Read the model definition and answer for the solid it produces. Units are mm, in the model's axes. Face numbers are marked on the shaded views. A direction names the side the tool comes from. Coordinates: 2 decimals unless noted, no trailing zeros. Order: outer loops, then holes, each group sorted by start corner. A loop starts at its lowest first (then second) coordinate and runs counter-clockwise, first axis right, second up. Notation, with made-up numbers: (4.25, 85) -> (33.25, 85) arc R20 cw to (33.25, 115) -> close; hole circle Ø10 at (39.25, -27.5). An arc over 180 degrees is marked (long way). Answer in a Markdown table with one row per item.
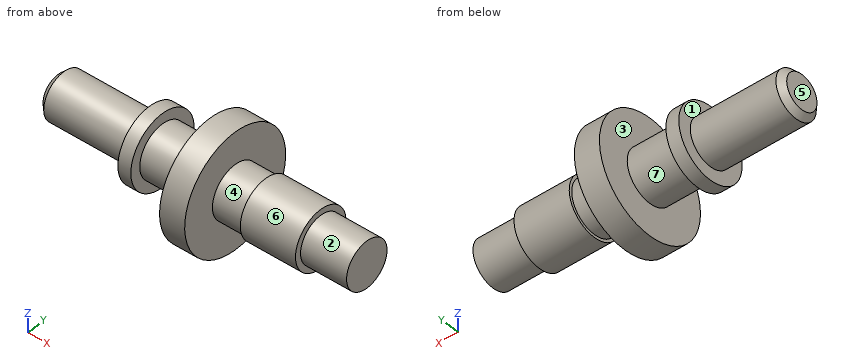
from build123d import *


with BuildPart() as part:
    # Model → Revolve1 (revolve)
    with BuildSketch(Plane.XY, mode=Mode.PRIVATE) as revolve1_sk:
        Polygon((49.51331086, -13.474001866), (49.517097509, -14.469395389), (57.517097509, -14.469395389), (57.517097509, -18.474001866), (3.884490088, -18.474001866), (3.884490088, -15.474001866), (4.884490088, -14.474001866), (11.769027201, -14.474001866), (19.769026262, -14.474001866), (19.769027201, -12.204912355), (22.015056766, -12.204912355), (22.015056766, -13.974001866), (30.280660424, -13.974001866), (30.280660424, -8.474001866), (34.643062355, -8.474001866), (34.643062355, -13.974001866), (39.923864692, -13.974001866), (39.923864692, -13.474001866), align=None)
    revolve(revolve1_sk.sketch.rotate(Axis((3.884490088, -18.474001866, 0), (-1, 0, 0)), 90), axis=Axis((3.884490088, -18.474001866, 0), (-1, 0, 0)))


solid = part.part
Q1. Consider line 1 (X direction, y = -20.75, z = -4.75); line 2 (X direction, y = -25.5, z = -1.75); line 3 (Z direction, x = 12, y = -20.5). Determine where each line is inside the solid, lowest interval first.
Outcome:
| item | result |
|---|---|
| line 1 | 19.77 to 22.02, 30.28 to 34.64 |
| line 2 | 30.28 to 34.64 |
| line 3 | -3.45 to 3.45 |
Q2. For the marked faces 1, 2 and 3, determine the directions among +Z, -Z, +X, -X, +Y, -Y from which every point of the face is accessible in a straight line to the end or side of a thin tool.
Outcome:
| item | result |
|---|---|
| face 1 | -X |
| face 2 | +X |
| face 3 | none |
Q3. The part is cut by section B-B (x = 15). Write down the section's boundary in (y, z), then the cut area to 3 significant figures.
Outcome:
| item | result |
|---|---|
| outline | circle Ø8 at (-18.47, 0) |
| area | 50.3 mm² |
Q4. Given pin 1 (2 mm diameter, centred on x = 19.5, z = -4, fed in from +Y); pin 2 (5 mm diameter, centred on x = 19, z = -4.5, fed in from -Y); pin 3 (10 mm diameter, centred on x = 40.5, z = 0, fed in from +Y), each flat-ended and moving along its own axis, determine where each tip first touches the part or whether it passes through.
Outcome:
| item | result |
|---|---|
| pin 1 | y = -12.99 |
| pin 2 | y = -24.37 |
| pin 3 | y = -13.47 |
Q5. The part is cut by section D-D (z = 8.75). Write down the section's boundary in (x, y), then the cut area to 3 significant figures.
Outcome:
| item | result |
|---|---|
| outline | (30.28, -23.32) -> (34.64, -23.32) -> (34.64, -13.63) -> (30.28, -13.63) -> close |
| area | 42.2 mm² |
Q6. For a pull along X with two mould halves and no side action, classify the marked faces 4, 5, 6 and 7 as pulls with the +X half, pulls with the -X half, needs draft (parallel to the pull), parting line crosses it, or undercut.
Outcome:
| item | result |
|---|---|
| face 4 | undercut |
| face 5 | pulls with the -X half |
| face 6 | needs draft |
| face 7 | undercut |
Q7. The part is cut by section C-C (x = 38.5). Write down the section's boundary in (y, z), then the cut area to 3 significant figures.
Outcome:
| item | result |
|---|---|
| outline | circle Ø9 at (-18.47, 0) |
| area | 63.6 mm² |
